The model under review builds one solid part; all positions refer to its coordinate system, in mm. A direction names the side the tool comes from. Give positions to 0.01 mm unless a question says otherwise; leave off trailing zeros. Order: outer loops, then holes, each group sorted by start corner. A loop starts at its lowest first (then second) coordinate and runs counter-clockwise, first axis right, second up. Notation, with made-up numbers: (74.5, 53) -> (125.5, 53) arc R20 cw to (125.5, 79) -> close; hole circle Ø8 at (-40, -1.75). An arc over 180 degrees is marked (long way). Use one line per item in the form item = value.
```python
from build123d import *

# Parameters (mm, degrees)
SKETCH1_R             = 27.5
BOSS_EXTRUDE1_DEPTH   = 325
SKETCH2_R             = 12.5
BOSS_EXTRUDE2_DEPTH   = 40
CHAMFER1_SIZE         = 1
SKETCH3_R             = 10
BOSS_EXTRUDE3_DEPTH   = 32
CHAMFER2_SIZE         = 1
CUT_EXTRUDE1_START    = -6.5
CUT_EXTRUDE1_DEPTH    = 10
M5_TAPPED_HOLE1_D     = 4.2
M5_TAPPED_HOLE1_DEPTH = 12.4
M5_TAPPED_HOLE1_TIP   = 1.2618073


with BuildPart() as part:
    # Sketch1 → Boss-Extrude1 (new, symmetric)
    with BuildSketch(Plane.XY):
        Circle(SKETCH1_R)
    extrude(amount=BOSS_EXTRUDE1_DEPTH, both=True)

    # Sketch2 → Boss-Extrude2 (add)
    with BuildSketch(Plane.XY.offset(325)):
        Circle(SKETCH2_R)
    boss_extrude2 = extrude(amount=BOSS_EXTRUDE2_DEPTH)

    # Mirror1: Boss-Extrude2 across plane
    add(boss_extrude2.mirror(Plane.XY))

    # Chamfer1
    chamfer1_edges = [part.edges().sort_by_distance(p)[0] for p in [
        (-12.5, 0, -365),
        (-27.5, 0, -325),
        (-27.5, 0, 325),
        (-12.5, 0, 365),
    ]]
    chamfer(chamfer1_edges, length=CHAMFER1_SIZE)

    # Sketch3 → Boss-Extrude3 (add)
    with BuildSketch(Plane.XY.offset(365)):
        Circle(SKETCH3_R)
    extrude(amount=BOSS_EXTRUDE3_DEPTH)

    # Chamfer2
    chamfer2_edges = [part.edges().sort_by_distance(p)[0] for p in [
        (-10, 0, 397),
    ]]
    chamfer(chamfer2_edges, length=CHAMFER2_SIZE)

    # Sketch4 → Cut-Extrude1 (cut)
    with BuildSketch(Plane(origin=(0, 0, 0), x_dir=(1, 0, 0), z_dir=(0, 1, 0)).offset(CUT_EXTRUDE1_START)):
        with BuildLine():
            Line((-3, -424.5), (-3, -369.5))
            ThreePointArc((-3, -369.5), (0, -366.5), (3, -369.5))
            Line((3, -369.5), (3, -424.5))
            ThreePointArc((3, -424.5), (0, -427.5), (-3, -424.5))
        make_face()
    extrude(amount=-CUT_EXTRUDE1_DEPTH, mode=Mode.SUBTRACT)

    # M5 Tapped Hole1
    with Locations(Plane.XY.offset(397)):
        with Locations((0, 0)):
            Hole(M5_TAPPED_HOLE1_D / 2, depth=M5_TAPPED_HOLE1_DEPTH)
            with Locations((0, 0, -(M5_TAPPED_HOLE1_DEPTH + M5_TAPPED_HOLE1_TIP / 2))):  # 118° drill point
                Cone(0, M5_TAPPED_HOLE1_D / 2, M5_TAPPED_HOLE1_TIP, mode=Mode.SUBTRACT)


solid = part.part
```
1. Add section A-A on z = 127.5. Give the boundary of the cut face in (x, y), then the cut area to 3 significant figures.
Values:
outline = circle Ø55 at (0, 0)
area = 2,380 mm^2
2. Tool access review of faces 1 (the face through (11.4, -5.5, -325)), 2 (the face through (-5.961, -26.846, 4.536)), 3 (the face through (5.38, 8.43, 380.28)): name each direction out of +Z, -Z, +X, -X, +Y, -Y from which nothing blocks a thin tool from reaching the whole face with its end or side.
Values:
face_1 = -Z
face_2 = +Z, -Z
face_3 = +Z
3. For pin 1 Ø6 at (x, z) = (16, -152) entering from -Y; pin 2 Ø4 at (x, y) = (19, 11.5) entering from -Z; pin 3 Ø2.5 at (y, z) = (-7.5, 378) entering from -X, all flat-tipped, find the tip position at first contact; note any pin that passes through.
Values:
pin_1 = -24.23
pin_2 = -325
pin_3 = -7.81
4. For L1, parallel to X at y = 0, z = 391.5; L2, parallel to Y at x = 0, z = 391; L3, parallel to Z at x = -15, y = 19.5, list the stretches that pass through material, from the lowest coordinate up.
Values:
L1 = -10 to -2.1, 2.1 to 10
L2 = -6.5 to -2.1, 2.1 to 10
L3 = -325 to 325
